Design review of the part built by this model. Coordinates are the model's own, in mm. Face numbers are marked on the shaded views. A direction names the side the tool comes from. Round coordinates to 2 decimals unless told otherwise and drop trailing zeros. Order: outer loops, then holes, each group sorted by start corner. A loop starts at its lowest first (then second) coordinate and runs counter-clockwise, first axis right, second up. Notation, with made-up numbers: (88, -28.75) - (125, -28.75) arc R19 ccw to (125, -22.75) - close; hole circle Ø3 at (-24, 46). An arc over 180 degrees is marked (long way). Write item = value, one per line.
from build123d import *


with BuildPart() as part:
    # Sketch1 → Revolve1 (revolve)
    with BuildSketch(Plane.XZ, mode=Mode.PRIVATE) as revolve1_sk:
        Polygon((12, 28), (12.5, 28), (12.5, 0), (17, 0), (17.5, 0.5), (17.5, 49.5), (17, 50), (12, 50), align=None)
    revolve(revolve1_sk.sketch.rotate(Axis((0, 0, 50), (0, 0, -1)), 180), axis=Axis((0, 0, 50), (0, 0, -1)))


solid = part.part
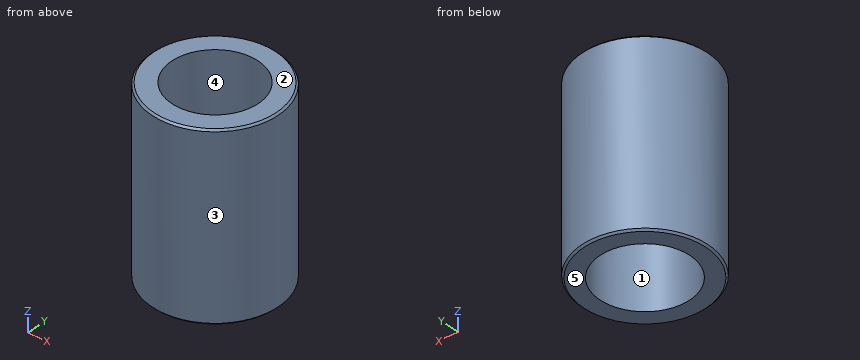
Item 1: Insertion check: P1, Ø5, axis at y = -13, z = 9.5, coming from the +X side; P2, Ø1, axis at y = -5.5, z = 25, coming from the -X side; P3, Ø10, axis at y = -6.5, z = 38, coming from the +X side; P4, Ø10, axis at x = 4, z = 9, coming from the +Y side. Each pin has a flat end and moves straight along its axis. Give the tip position at first contact, or say it passes through.
Data:
P1 = 14
P2 = -16.77
P3 = 17.44
P4 = 17.5
Item 2: For the marked faces 1 and 2, list the 3-axis set-ups (+Z, -Z, +X, -X, +Y, -Y) from which the entire face can be reached by the end or side of a thin tool; tool diameter is ignored.
Data:
face_1 = -Z
face_2 = +Z, +X, -X, +Y, -Y
Item 3: Take a section at A-A, the plane y = 0. State the section outline as (x, z) points, and give its area (4 significant figures).
Data:
outline = (-17.5, 0.5) - (-17, 0) - (-12.5, 0) - (-12.5, 28) - (-12, 28) - (-12, 50) - (-17, 50) - (-17.5, 49.5) - close; (12, 28) - (12.5, 28) - (12.5, 0) - (17, 0) - (17.5, 0.5) - (17.5, 49.5) - (17, 50) - (12, 50) - close
area = 521.5 mm2
Item 4: Take a section at D-D, the plane z = 33. State the section outline as (x, y) points.
Data:
outline = circle Ø35 at (0, 0); hole circle Ø24 at (0, 0)
Item 5: For line 1 along Y through (x, z) = (0, 37); line 2 along Y through (x, z) = (0.5, 24); line 3 along X through (y, z) = (4.5, 37), list the stretches that pass through material, from the lowest coordinate up. Write a range as [from, to].
Data:
line_1 = [-17.5, -12], [12, 17.5]
line_2 = [-17.49, -12.49], [12.49, 17.49]
line_3 = [-16.91, -11.12], [11.12, 16.91]
Item 6: Take a section at C-C, the plane z = 10. State the section outline as (x, y) points, and give its area (3 significant figures).
Data:
outline = circle Ø35 at (0, 0); hole circle Ø25 at (0, 0)
area = 471 mm2
Item 7: The part is to be moulded in two halves that separate along X. For the marked faces 3, 4 and 5, say which applies: +X half, -X half, draft (parallel to the pull), parting line (faces both ways), or undercut.
Data:
face_3 = parting line
face_4 = undercut
face_5 = draft
